Can you work these out from the model? Positions are in its coordinate system, mm. Face numbers are marked on the shaded views. A direction names the side the tool comes from. Give positions to 0.01 mm unless a question says otherwise; leave off trailing zeros. Loops run counter-clockwise (first coordinate to the right, second up) from the corner with the lowest first, then second, coordinate; pieces in that order, holes last. Notation, with made-up numbers: M -29,67 L 11,67 A32 cw 11,102 Z; hole C 32.5,-32 d8. An arc over 180 degrees is marked long. Use CSV: the item, a comma, the result in double quotes.
from build123d import *

# Parameters (mm, degrees)
SKETCH_1_W             = 60
SKETCH_1_H             = 140
BOSS_EXTRUDE_1_DEPTH   = 10
SKETCH_4_W             = 10
SKETCH_4_H             = 30
CUT_EXTRUDE_1_DEPTH    = 77.811457479
LINEAR_PATTERN_2_COUNT = 3
LINEAR_PATTERN_2_PITCH = 60
M5_TAPPED_HOLE_3_D     = 4.2
M5_TAPPED_HOLE_3_DEPTH = 12.4
M5_TAPPED_HOLE_3_TIP   = 1.2618073


with BuildPart() as part:
    # Sketch 1 → Boss-Extrude 1 (new body)
    with BuildSketch(Plane(origin=(0, 0, 0), x_dir=(0, 0, -1), z_dir=(1, 0, 0))):
        Rectangle(SKETCH_1_W, SKETCH_1_H)
    extrude(amount=BOSS_EXTRUDE_1_DEPTH)

    # Sketch 4 → Cut-Extrude 1 (cut, through all)
    with BuildSketch(Plane.ZY):
        with Locations((25, 0)):
            Rectangle(SKETCH_4_W, SKETCH_4_H)
    extrude(amount=-CUT_EXTRUDE_1_DEPTH, mode=Mode.SUBTRACT)

    # Sketch 5 → M5 Tapped Hole 2 (revolve, cut)
    with BuildSketch(Plane(origin=(5, 60, -30), x_dir=(0, 1, 0), z_dir=(1, 0, 0))):
        Polygon((0, 0), (0, 13.6618073), (2.1, 12.4), (2.1, 0), align=None)
    m5_tapped_hole_2 = revolve(axis=Axis((5, 60, -36.35), (0, 0, 1)), mode=Mode.SUBTRACT)

    # Linear Pattern 2: M5 Tapped Hole 2 ×3
    with Locations(*[(0, -i * LINEAR_PATTERN_2_PITCH, 0) for i in range(1, LINEAR_PATTERN_2_COUNT)]):
        add(m5_tapped_hole_2, mode=Mode.SUBTRACT)

    # M5 Tapped Hole 3
    with Locations(Plane.XY.offset(30)):
        with Locations((5, -60), (5, -30), (5, 30), (5, 60)):
            Hole(M5_TAPPED_HOLE_3_D / 2, depth=M5_TAPPED_HOLE_3_DEPTH)
            with Locations((0, 0, -(M5_TAPPED_HOLE_3_DEPTH + M5_TAPPED_HOLE_3_TIP / 2))):  # 118° drill point
                Cone(0, M5_TAPPED_HOLE_3_D / 2, M5_TAPPED_HOLE_3_TIP, mode=Mode.SUBTRACT)


solid = part.part
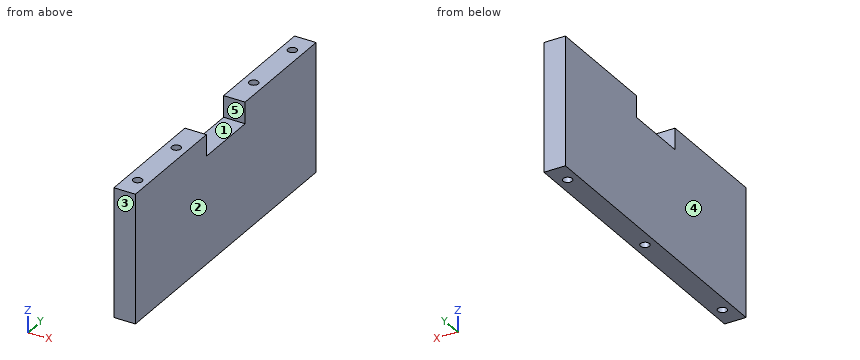
Q1. If we mould it in two halves opening along Y, with no side actions, what happens to the marked faces 1, 2 and 3? For each: released by +Y, released by -Y, zero draft, split by the parting line, or undercut.
Model answer:
face 1,"undercut"
face 2,"zero draft"
face 3,"released by -Y"
Q2. I want a section at D-D, the plane y = 6. Please give me the cut outline in (x, z), then the cut area to 3 significant figures.
Model answer:
outline,"M 0,-30 L 10,-30 L 10,20 L 0,20 Z"
area,"500 mm2"
Q3. For the marked faces 4 and 5, which set-ups out of +Z, -Z, +X, -X, +Y, -Y let a thin tool reach every point of the face, with its end or its side?
Model answer:
face 4,"+Z, -Z, -X, +Y, -Y"
face 5,"+Z, +X, -X"
Q4. I want a section at B-B, the plane z = -19. Please give me the cut outline in (x, y), then the cut area to 3 significant figures.
Model answer:
outline,"M 0,-70 L 10,-70 L 10,70 L 0,70 Z; hole C 5,-60 d4.2; hole C 5,0 d4.2; hole C 5,60 d4.2"
area,"1,360 mm2"
Q5. I'm going to push flat-ended pins straight in: P1, Ø2.5, axis at x = 5, y = 0, coming from the -Z side; P2, Ø3, axis at x = 4.5, y = 3, coming from the +Z side; P3, Ø3.5, axis at x = 5, y = 60, coming from the -Z side. Where does each tip first touch, or does it pass through?
Model answer:
P1,"z = -17.09"
P2,"z = 20"
P3,"z = -17.39"
Q6. I want a section at A-A, the plane z = 21.5. Please give me the cut outline in (x, y), then the cut area to 3 significant figures.
Model answer:
outline,"M 0,-70 L 10,-70 L 10,-15 L 0,-15 Z; M 0,15 L 10,15 L 10,70 L 0,70 Z; hole C 5,-60 d4.2; hole C 5,-30 d4.2; hole C 5,30 d4.2; hole C 5,60 d4.2"
area,"1,040 mm2"
Q7. Please list where these lines run through material, in increasing order: L1, parallel to Y at x = 5, z = -27.25; L2, parallel to Y at x = 5, z = 23.5; L3, parallel to X at y = 60, z = 24. Write a range as from..to.
Model answer:
L1,"-70..-62.1, -57.9..-2.1, 2.1..57.9, 62.1..70"
L2,"-70..-62.1, -57.9..-32.1, -27.9..-15, 15..27.9, 32.1..57.9, 62.1..70"
L3,"0..2.9, 7.1..10"
Q8. I want a section at C-C, the plane x = 1.25. Please give me the cut outline in (y, z).
Model answer:
outline,"M -70,-30 L 70,-30 L 70,30 L 15,30 L 15,20 L -15,20 L -15,30 L -70,30 Z"
